from build123d import *

# Parameters (mm, degrees)
CHAMFER1_SIZE = 0.5


with BuildPart() as part:
    # Sketch1 → Revolve1 (revolve)
    with BuildSketch(Plane.XY, mode=Mode.PRIVATE) as revolve1_sk:
        Polygon((74.023669398, -131.5), (74.023669398, -118.5), (80.273669398, -118.5), (80.273669398, -127.5), (79.773669398, -127.5), (79.773669398, -128.5), (82.023669398, -128.5), (82.023669398, -131.5), align=None)
    revolve(revolve1_sk.sketch.rotate(Axis((74.023669398, -118.5, 0), (0, -1, 0)), 90), axis=Axis((74.023669398, -118.5, 0), (0, -1, 0)))

    # Chamfer1
    chamfer1_edges = [part.edges().sort_by_distance(p)[0] for p in [
        (74.023669398, -131.5, -8),
        (74.023669398, -128.5, -8),
        (74.023669398, -118.5, -6.25),
    ]]
    chamfer(chamfer1_edges, length=CHAMFER1_SIZE)


solid = part.part
Model file for the job. Use its own axes, mm. A direction names the side the tool comes from. Give positions to 0.01 mm unless a question says otherwise; leave off trailing zeros. Order: outer loops, then holes, each group sorted by start corner. A loop starts at its lowest first (then second) coordinate and runs counter-clockwise, first axis right, second up. Notation, with made-up numbers: M -39.75,9.25 L 9.25,9.25 A31 ccw 9.25,43.25 Z; hole C 64.25,18.25 d3. An arc over 180 degrees is marked long. Put each result on its own line as item: value. Start each with the question number.
(1) Drill centre lines: L1, parallel to Y at x = 79.25, z = 5.25; L2, parallel to Y at x = 68, z = -1; L3, parallel to X at y = -123.5, z = 0. Where is each one in solid material? Low to high. Write a range as [from, to].
(2) Band-saw the part on B-B on y = -121. Give the cut face in (x, z).
(3) Pin check, flat tips, straight feed: pin 1 Ø4 at (x, y) = (80, -121.5) entering from +Z; pin 2 Ø1.5 at (y, z) = (-124.5, 6) entering from -X; pin 3 Ø5 at (y, z) = (-126.5, -4) entering from -X; pin 4 Ø5 at (x, y) = (76, -130) entering from -Z. Stop position of each tip, or through.
(4) Pull direction Y, two halves, no side cores. Call faces 3 (the face through (80, -128.5, 2)), 4 (the face through (80.125, -123.31, -1.355)), 5 (the face through (74, -118.5, 0)), 6 (the face through (74, -131.5, 0)): released by +Y, released by -Y, zero draft, split by the parting line, or undercut.
(5) Band-saw the part on A-A on z = 0. Give the cut face in (x, y).
(6) Tool access for faces 1 (the face through (81.833, -130.014, -1.734)), 2 (the face through (69.175, -128.007, 3.091)): list every direction of +Z, -Z, +X, -X, +Y, -Y with a clear straight run to the whole face (end or side of a thin tool).
Results below:
1. L1: y = [-131.5, -128.5]
1. L2: y = [-131.5, -128.5], [-127.5, -118.86]
1. L3: x = [67.77, 80.27]
2. outline: C 74.02,0 d12.5
3. pin 1: stops at z = 4.82
3. pin 2: stops at x = 70.63
3. pin 3: stops at x = 66.83
3. pin 4: stops at z = -8
4. face 3: undercut
4. face 4: zero draft
4. face 5: released by +Y
4. face 6: released by -Y
5. outline: M 66.02,-131 L 66.52,-131.5 L 81.52,-131.5 L 82.02,-131 L 82.02,-129 L 81.52,-128.5 L 79.77,-128.5 L 79.77,-127.5 L 80.27,-127.5 L 80.27,-119 L 79.77,-118.5 L 68.27,-118.5 L 67.77,-119 L 67.77,-127.5 L 68.27,-127.5 L 68.27,-128.5 L 66.52,-128.5 L 66.02,-129 Z
6. face 1: +Y, -Y
6. face 2: none
